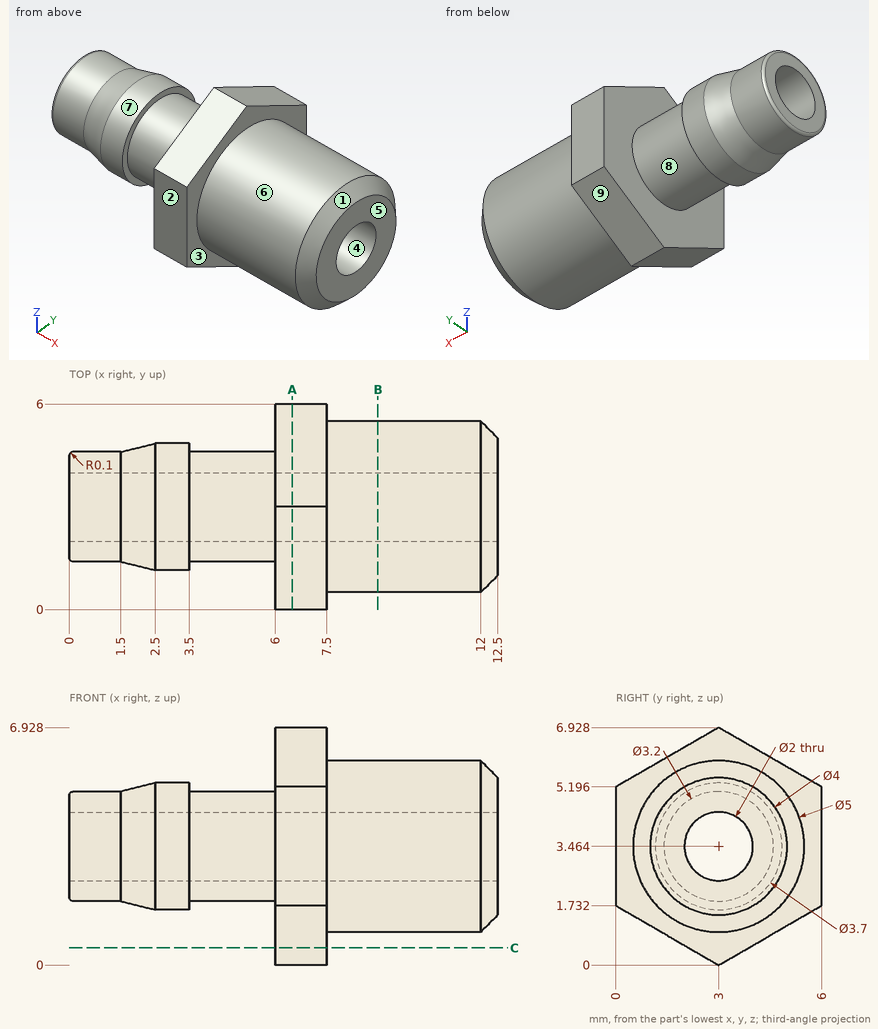
Source: three-view drawing plus pictorial views. Frame: mm from the lowest corner of the part. A direction names the side the tool comes from. Give positions to 0.01 mm unless a question says otherwise; leave off trailing zeros. Order: outer loops, then holes, each group sorted by start corner. A loop starts at its lowest first (then second) coordinate and runs counter-clockwise, first axis right, second up. Notation, with made-up numbers: (64.25, 16.5) -> (94.25, 16.5) arc R23 ccw to (94.25, 49.5) -> close; hole circle Ø2 at (15, 10). An arc over 180 degrees is marked (long way). Use a Markdown table: item, result.
Q1. Section B-B (x = 9). Return the cut outline in (y, z), and give its area (3 significant figures).
A:
| item | result |
|---|---|
| outline | circle Ø5 at (3, 3.46); hole circle Ø2 at (3, 3.46) |
| area | 16.5 mm^2 |
Q2. Pull-direction query (Y, two-part tool) for the marked faces 1, 2, 3 and 4; classes: +Y half, -Y half, draft (parallel to the pull), parting line (faces both ways), or undercut.
A:
| item | result |
|---|---|
| face 1 | parting line |
| face 2 | -Y half |
| face 3 | draft |
| face 4 | undercut |
Q3. First-contact query: P1, Ø3, axis at x = 11, z = 1, coming from the +Y side; P2, Ø1, axis at x = 2.5, z = 5.5, coming from the +Y side; P3, Ø1.5, axis at x = 2.5, y = 4.5, coming from the -Z side; P4, Ø1.2, axis at y = 3, z = 3.46, coming from the -X side. Flat tips, straight axial feed; report the tip coordinate or a pass-through.
A:
| item | result |
|---|---|
| P1 | y = 5.31 |
| P2 | y = 4.03 |
| P3 | z = 1.77 |
| P4 | through |
Q4. Section A-A (x = 6.5). Return the cut outline in (y, z).
A:
| item | result |
|---|---|
| outline | (0, 1.73) -> (3, 0) -> (6, 1.73) -> (6, 5.2) -> (3, 6.93) -> (0, 5.2) -> close; hole circle Ø2 at (3, 3.46) |
Q5. Section C-C (z = 0.5). Return the cut outline in (x, y).
A:
| item | result |
|---|---|
| outline | (6, 2.13) -> (7.5, 2.13) -> (7.5, 3.87) -> (6, 3.87) -> close |
Q6. Material intervals for line 1 (Z direction, x = 7.75, y = 4.5) (1 decimal); line 2 (X direction, y = 3.5, z = 6); line 3 (X direction, y = 4.5, z = 3.25), sorted ascending. Write a range as [from, to].
A:
| item | result |
|---|---|
| line 1 | [1.5, 5.5] |
| line 2 | [6, 7.5] |
| line 3 | [0, 12.5] |
Q7. Access query for the marked faces 5, 6, 7, 8 and 9. Directions: +Z, -Z, +X, -X, +Y, -Y. A direction counts if a zero-diameter tool reaches every point of the face in a straight line with its end or side. Return the directions, or none.
A:
| item | result |
|---|---|
| face 5 | +Z, -Z, +X, +Y, -Y |
| face 6 | +X |
| face 7 | -X |
| face 8 | none |
| face 9 | -Z, +X, -X, +Y |
